```python
from build123d import *

# Parameters (mm, degrees)
SKETCH3_OUTSIDE_W  = 22.05
SKETCH3_OUTSIDE_H  = 22.05
CUT_EXTRUDE1_DEPTH = 5


with BuildPart() as part:
    # Sketch1 → Revolve1 (revolve)
    with BuildSketch(Plane.XY, mode=Mode.PRIVATE) as revolve1_sk:
        Polygon((1.45, 0), (2.3, 0), (2.5, 0.2), (2.5, 3), (2, 3), (2, 3.5), (4.3, 3.5), (4.5, 3.7), (4.5, 8.5), (5.5, 9.5), (5.5, 11.5), (5.8, 11.5), (6, 11.7), (6, 20.3), (5.8, 20.5), (4.75, 20.5), (4.75, 21.5), (5.2, 21.5), (5.2, 33.8), (5, 34), (4, 34), (4, 35), (5, 35), (5, 36.3), (4.8, 36.5), (2.2, 36.5), (2, 36.3), (2, 5.75), (1.25, 5), (1.25, 0.2), align=None)
    revolve(revolve1_sk.sketch.rotate(Axis((0, 0, 0), (0, 1, 0)), 90), axis=Axis((0, 0, 0), (0, 1, 0)))

    # Sketch3 outside → Cut-Extrude1 (cut)
    with BuildSketch(Plane.XZ.offset(-3.5)):
        Rectangle(SKETCH3_OUTSIDE_W, SKETCH3_OUTSIDE_H)
        Polygon((2.309401077, -4), (4.618802154, 0), (2.309401077, 4), (-2.309401077, 4), (-4.618802154, 0), (-2.309401077, -4), align=None, mode=Mode.SUBTRACT)
    extrude(amount=-CUT_EXTRUDE1_DEPTH, mode=Mode.SUBTRACT)


solid = part.part
```
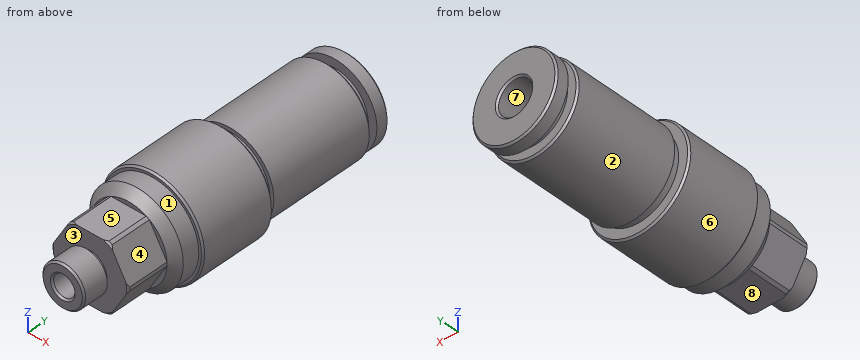
Input: part model. Units: mm. Frame: model coordinates. Face numbers are marked on the shaded views. A direction names the side the tool comes from. Coordinates: 2 decimals unless noted, no trailing zeros. Loops run counter-clockwise (first coordinate to the right, second up) from the corner with the lowest first, then second, coordinate; pieces in that order, holes last. Notation, with made-up numbers: M 77.25,-39 L 99.25,-39 A30 ccw 99.25,0 Z; hole C 88,60.25 d9. An arc over 180 degrees is marked long. Use a Markdown table: item, result. Add a question column.
1) Pin query (flat end, axial travel): P1, Ø2, axis at x = 0, z = 0, coming from the +Y side; P2, Ø1.6, axis at x = -4, z = -1.5, coming from the -Y side; P3, Ø2, axis at x = 0, y = 6.5, coming from the +Z side; P4, Ø4, axis at x = 1.5, y = 23, coming from the +Z side. Return the tip coordinate at first contact, or that it passes through.
2) Section A-A, the plane y = 25.5. Return the cut outline in (x, z), plus the area to 3 significant figures.
3) Section B-B, the plane y = 13. Return the cut outline in (x, z), plus the area to 3 significant figures.
4) Draft query along X for the marked faces 6, 7 and 8. Return one class per face: +X half, -X half, draft (parallel to the pull), parting line (faces both ways), or undercut.
5) Set-up query: the marked faces 1, 2, 3, 4 and 5. Return all of +Z, -Z, +X, -X, +Y, -Y with unobstructed straight access to the full face (end or side cutting, diameter ignored); none if empty.
6) Line query: L1, parallel to X at y = 1.6, z = 0; L2, parallel to X at y = 25.5, z = 0; L3, parallel to Y at x = 2.75, z = -3.5. Output: solid intervals per line, ascending. Write a range as from..to.
Answer below:
| question | item | result |
|---|---|---|
| 1 | P1 | through |
| 1 | P2 | y = 3.5 |
| 1 | P3 | z = 4 |
| 1 | P4 | z = 5.2 |
| 2 | outline | C 0,0 d10.4; hole C 0,0 d4 |
| 2 | area | 72.4 mm2 |
| 3 | outline | C 0,0 d12; hole C 0,0 d4 |
| 3 | area | 101 mm2 |
| 4 | face 6 | parting line |
| 4 | face 7 | undercut |
| 4 | face 8 | draft |
| 5 | face 1 | -Y |
| 5 | face 2 | +Y |
| 5 | face 3 | none |
| 5 | face 4 | +Z, +X, -Y |
| 5 | face 5 | +Z, +X, -X, -Y |
| 6 | L1 | -2.5..-1.25, 1.25..2.5 |
| 6 | L2 | -5.2..-2, 2..5.2 |
| 6 | L3 | 8.5..34, 35..36.5 |
